For this review, take the finished solid that the model builds, in its own axes (mm). Face numbers are marked on the shaded views. Give positions to 0.01 mm unless a question says otherwise; leave off trailing zeros. Loops run counter-clockwise (first coordinate to the right, second up) from the corner with the lowest first, then second, coordinate; pieces in that order, holes last.
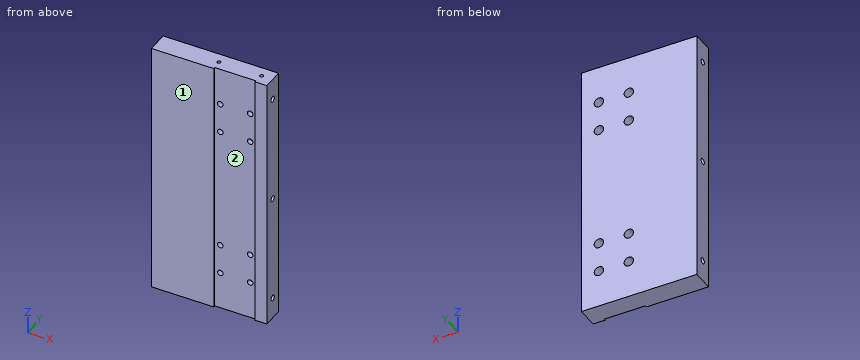
```python
from build123d import *

# Parameters (mm, degrees)
SKETCH_1_W                   = 135
SKETCH_1_H                   = 300
EXTRUDE_1_DEPTH              = 25
SKETCH_2_W                   = 48
SKETCH_2_H                   = 2
CUT_EXTRUDE_1_DEPTH          = 309.514586365
HOLE_WIZARD_M8_1_AT_2_COUNT  = 2
HOLE_WIZARD_M8_1_AT_2_PITCH  = 250
HOLE_WIZARD_M8_1_AT_3_COUNT  = 2
HOLE_WIZARD_M8_1_AT_3_PITCH  = 125
HOLE_WIZARD_M6_1_D           = 6.6
HOLE_WIZARD_M6_1_CBORE_D     = 11
HOLE_WIZARD_M6_1_CBORE_DEPTH = 16.8
HOLE_WIZARD_M5_1_D           = 4.2
HOLE_WIZARD_M5_1_DEPTH       = 12.4
HOLE_WIZARD_M5_1_TIP         = 1.2618073


with BuildPart() as part:
    # 草图1 → 凸台-拉伸1 (new body)
    with BuildSketch(Plane(origin=(0, 0, 0), x_dir=(1, 0, 0), z_dir=(0, 1, 0))):
        Rectangle(SKETCH_1_W, SKETCH_1_H)
    extrude(amount=EXTRUDE_1_DEPTH)

    # 草图2 → 切除-拉伸1 (cut, through all)
    with BuildSketch(Plane.XY.offset(150)):
        with Locations((29.5, 1)):
            Rectangle(SKETCH_2_W, SKETCH_2_H)
    extrude(amount=-CUT_EXTRUDE_1_DEPTH, mode=Mode.SUBTRACT)

    # 草图6 → M8 螺纹孔1 (revolve, cut)
    with BuildSketch(Plane(origin=(-67.5, 12.5, -125), x_dir=(0, 0, 1), z_dir=(0, 1, 0))):
        Polygon((0, 0), (0, 21.792926105), (3.4, 19.75), (3.4, 0), align=None)
    hole_wizard_m8_1 = revolve(axis=Axis((-73.85, 12.5, -125), (1, 0, 0)), mode=Mode.SUBTRACT)

    # M8 螺纹孔1 at 2: M8 螺纹孔1 ×2
    with Locations(*[(0, 0, i * HOLE_WIZARD_M8_1_AT_2_PITCH) for i in range(1, HOLE_WIZARD_M8_1_AT_2_COUNT)]):
        add(hole_wizard_m8_1, mode=Mode.SUBTRACT)

    # M8 螺纹孔1 at 3: M8 螺纹孔1 ×2
    with Locations(*[(0, 0, i * HOLE_WIZARD_M8_1_AT_3_PITCH) for i in range(1, HOLE_WIZARD_M8_1_AT_3_COUNT)]):
        add(hole_wizard_m8_1, mode=Mode.SUBTRACT)

    # 镜向1: M8 螺纹孔1 across plane
    add(hole_wizard_m8_1.mirror(Plane(origin=(0, 0, 0), x_dir=(0, 0, 1), z_dir=(1, 0, 0))), mode=Mode.SUBTRACT)

    # 镜向1 copy 1 sketch → 镜向1 copy 1 (revolve, cut)
    with BuildSketch(Plane(origin=(67.5, 12.5, 125), x_dir=(0, 0, 1), z_dir=(0, 1, 0))):
        Polygon((0, 0), (0, -21.792926105), (3.4, -19.75), (3.4, 0), align=None)
    revolve(axis=Axis((73.85, 12.5, 125), (1, 0, 0)), mode=Mode.SUBTRACT)

    # 镜向1 copy 2 sketch → 镜向1 copy 2 (revolve, cut)
    with BuildSketch(Plane(origin=(67.5, 12.5, 0), x_dir=(0, 0, 1), z_dir=(0, 1, 0))):
        Polygon((0, 0), (0, -21.792926105), (3.4, -19.75), (3.4, 0), align=None)
    revolve(axis=Axis((73.85, 12.5, 0), (1, 0, 0)), mode=Mode.SUBTRACT)

    # M6 六角圆柱头螺钉的柱形沉头孔1 (through all)
    with Locations(Plane(origin=(0, 25, 0), x_dir=(1, 0, 0), z_dir=(0, 1, 0))):
        with Locations((12, -71.2), (47, -71.2), (47, -106.2), (12, -106.2), (12, 71.2), (12, 106.2), (47, 106.2), (47, 71.2)):
            CounterBoreHole(HOLE_WIZARD_M6_1_D / 2, HOLE_WIZARD_M6_1_CBORE_D / 2, HOLE_WIZARD_M6_1_CBORE_DEPTH)

    # M5 螺纹孔1
    with Locations(Plane.XY.offset(150)):
        with Locations((4.5, 12.5), (54.5, 12.5)):
            Hole(HOLE_WIZARD_M5_1_D / 2, depth=HOLE_WIZARD_M5_1_DEPTH)
            with Locations((0, 0, -(HOLE_WIZARD_M5_1_DEPTH + HOLE_WIZARD_M5_1_TIP / 2))):  # 118° drill point
                Cone(0, HOLE_WIZARD_M5_1_D / 2, HOLE_WIZARD_M5_1_TIP, mode=Mode.SUBTRACT)


solid = part.part
```
Item 1: The part is to be moulded in two halves that separate along X. For the marked faces 1 and 2, say which applies: released by +X, released by -X, zero draft, split by the parting line, or undercut.
Answer:
face 1: zero draft
face 2: undercut
Item 2: For L1, parallel to X at y = 21.75, z = -106.2; L2, parallel to Z at x = 56.5, y = 12.5; L3, parallel to Z at x = -59.75, y = 12.5, list the stretches that pass through material, from the lowest coordinate up.
Answer:
L1: x = -67.5 to 6.5, 17.5 to 41.5, 52.5 to 67.5
L2: z = -150 to -128.4, -121.6 to -3.4, 3.4 to 121.6, 128.4 to 137.54
L3: z = -150 to -128.4, -121.6 to -3.4, 3.4 to 121.6, 128.4 to 150
Item 3: Take a section at A-A on z = -106.2. Give the boundary of the cut face in (x, y), and give its area (3 significant figures).
Answer:
outline: (-67.5, 0) - (5.5, 0) - (5.5, 2) - (8.7, 2) - (8.7, 8.2) - (6.5, 8.2) - (6.5, 25) - (-67.5, 25) - close; (15.3, 2) - (43.7, 2) - (43.7, 8.2) - (41.5, 8.2) - (41.5, 25) - (17.5, 25) - (17.5, 8.2) - (15.3, 8.2) - close; (50.3, 2) - (53.5, 2) - (53.5, 0) - (67.5, 0) - (67.5, 25) - (52.5, 25) - (52.5, 8.2) - (50.3, 8.2) - close
area: 2,830 mm2
Item 4: Take a section at C-C on x = 12. State how many separate pieces and enclosed holes the cut face has, and give its area (3 significant figures).
Answer:
separate pieces: 5
enclosed holes: 0
area: 6,000 mm2
Item 5: Clearance check with flat-ended pins moving along their axes: pin 1 Ø4 at (x, y) = (54.5, 12.5) entering from +Z; pin 2 Ø3.5 at (x, z) = (13, 107) entering from +Y; pin 3 Ø3.5 at (x, z) = (44.5, 69.5) entering from +Y; pin 4 Ø10.5 at (x, z) = (47, 106.2) entering from -Y. State where each tip first meets the part, or that it passes through.
Answer:
pin 1: stops at z = 137.54
pin 2: passes through
pin 3: stops at y = 8.2
pin 4: stops at y = 2
Item 6: Take a section at B-B on z = -29. Give the boundary of the cut face in (x, y), and give its area (3 significant figures).
Answer:
outline: (-67.5, 0) - (5.5, 0) - (5.5, 2) - (53.5, 2) - (53.5, 0) - (67.5, 0) - (67.5, 25) - (-67.5, 25) - close
area: 3,280 mm2
